Here's how the part is built. I have some questions about the finished solid (model axes, mm). A direction names the side the tool comes from. Round coordinates to 2 decimals unless told otherwise and drop trailing zeros. Write each loop counter-clockwise with the first axis right and the second up, starting at its lowest first coordinate (ties: lowest second). Pieces come first, ordered by that corner, then holes. Notation, with made-up numbers: (70, 38.5) -> (112, 38.5) arc R14 cw to (112, 44.5) -> close; hole circle Ø9 at (15.25, -31.5). An arc over 180 degrees is marked (long way). Answer in a Markdown table with one row per item.
from build123d import *

# Parameters (mm, degrees)
SKETCH_1_W          = 30
SKETCH_1_H          = 50
SKETCH_1_W_2        = 24
SKETCH_1_H_2        = 44
EXTRUDE_1_DEPTH     = 900
SKETCH_2_R          = 10
CUT_EXTRUDE_2_DEPTH = 900
EXTRUDE_2_DEPTH     = 50
SKETCH_4_W          = 30
SKETCH_4_H          = 50
SKETCH_4_W_2        = 24
SKETCH_4_H_2        = 44
EXTRUDE_3_DEPTH     = 15
EXTRUDE_4_DEPTH     = 50


with BuildPart() as part:
    # 草图1 → 凸台-拉伸1 (new body)
    with BuildSketch(Plane.XY):
        with Locations((15, 25)):
            Rectangle(SKETCH_1_W, SKETCH_1_H)
        with Locations((15, 25)):
            Rectangle(SKETCH_1_W_2, SKETCH_1_H_2, mode=Mode.SUBTRACT)
    extrude(amount=EXTRUDE_1_DEPTH)

    # 草图2 → 切除-拉伸2 (cut)
    with BuildSketch(Plane(origin=(0, 50, 0), x_dir=(1, 0, 0), z_dir=(0, 1, 0))):
        with Locations(Location((15, -15, 0), (0, 0, 270))):
            Circle(SKETCH_2_R)
        with BuildLine():
            ThreePointArc((0, -15), (4.393398282, -4.393398282), (15, 0))
            Line((15, 0), (0, 0))
            Line((0, 0), (0, -15))
        make_face()
        with BuildLine():
            Line((30, 0), (15, 0))
            ThreePointArc((15, 0), (25.606601718, -4.393398282), (30, -15))
            Line((30, -15), (30, 0))
        make_face()
    extrude(amount=-CUT_EXTRUDE_2_DEPTH, mode=Mode.SUBTRACT)

    # 草图3 → 凸台-拉伸2 (add)
    with BuildSketch(Plane(origin=(0, 50, 0), x_dir=(1, 0, 0), z_dir=(0, 1, 0))):
        with BuildLine():
            Line((2, -15), (0, -15))
            ThreePointArc((0, -15), (15, 0), (30, -15))
            Line((30, -15), (28, -15))
            ThreePointArc((28, -15), (15, -2), (2, -15))
        make_face()
    extrude(amount=-EXTRUDE_2_DEPTH)

    # 草图4 → 凸台-拉伸3 (add)
    with BuildSketch(Plane.XY.offset(900)):
        with Locations((15, 25)):
            Rectangle(SKETCH_4_W, SKETCH_4_H)
        with Locations((15, 25)):
            Rectangle(SKETCH_4_W_2, SKETCH_4_H_2, mode=Mode.SUBTRACT)
    extrude(amount=EXTRUDE_3_DEPTH)

    # 草图5 → 凸台-拉伸4 (add)
    with BuildSketch(Plane(origin=(0, 50, 0), x_dir=(1, 0, 0), z_dir=(0, 1, 0))):
        with BuildLine():
            Line((-12.2207709, -920.098671199), (-8.128726759, -920.098671199))
            ThreePointArc((-8.128726759, -920.098671199), (15, -914.491908276), (38.128726759, -920.098671199))
            Line((38.128726759, -920.098671199), (42.2207709, -920.098671199))
            ThreePointArc((42.2207709, -920.098671199), (15, -912.491908276), (-12.2207709, -920.098671199))
        make_face()
    extrude(amount=-EXTRUDE_4_DEPTH)


solid = part.part
1) I want a section at A-A, the plane z = 600. List the corners of the cut face in (x, y) for me.
Response:
| item | result |
|---|---|
| outline | (0, 0) -> (30, 0) -> (30, 50) -> (0, 50) -> close; hole (3, 3) -> (27, 3) -> (27, 47) -> (3, 47) -> close |
2) For pin 1 (5 mm diameter, centred on x = 21.5, y = 18.5, fed in from +Z); pin 2 (23 mm diameter, centred on x = 15, z = 15, fed in from -Y); pin 3 (2 mm diameter, centred on x = 11, y = 18, fed in from +Z); pin 4 (12 mm diameter, centred on y = 16.5, z = 594.5, fed in from +X), each with a flat end and sliding along its axis, tell me the tip position at first contact or that it passes through.
Response:
| item | result |
|---|---|
| pin 1 | stops at z = 915.3 |
| pin 2 | stops at y = 0 |
| pin 3 | stops at z = 914.74 |
| pin 4 | stops at x = 30 |
3) We'd pull the mould along Y, two halves only. Please class faces 1 (the face through (15, 0, 454)), 2 (the face through (15, 3, 452)): +Y half, -Y half, draft (parallel to the pull), parting line (faces both ways), or undercut.
Response:
| item | result |
|---|---|
| face 1 | -Y half |
| face 2 | undercut |
4) Which directions (+Z, -Z, +X, -X, +Y, -Y) give clear straight access to the entire face, cutting with the end or side of a thin tool? Please do faces 3 (the face through (0, 25, 459)), 4 (the face through (18, 48.52, 24.54)), 5 (the face through (15.169, 25.308, 912.492)), 6 (the face through (30, 25, 459)).
Response:
| item | result |
|---|---|
| face 3 | -Z, -X, +Y, -Y |
| face 4 | +Y, -Y |
| face 5 | none |
| face 6 | -Z, +X, +Y, -Y |
5) I want a section at B-B, the plane y = 15.5. List the corners of the cut face in (x, z) for me, and give its area (3 significant figures).
Response:
| item | result |
|---|---|
| outline | (-12.22, 920.1) arc R52.51 ccw to (0, 914.68) -> (0, 15) arc R15 ccw to (30, 15) -> (30, 914.68) arc R52.51 ccw to (42.22, 920.1) -> (38.13, 920.1) arc R50.51 cw to (-8.13, 920.1) -> close; hole (3, 10) arc R13 ccw to (27, 10) -> (27, 913.88) arc R52.51 cw to (3, 913.88) -> close |
| area | 5,600 mm^2 |
6) I need wall thicknesses on line 1 (X direction, y = 32.5, z = 603); line 2 (Y direction, x = 10, z = 633.5); line 3 (X direction, y = 0.8, z = 15). Which ranges of each line are inside material? Lowest first, please. Write a range as [from, to].
Response:
| item | result |
|---|---|
| line 1 | x = [0, 3], [27, 30] |
| line 2 | y = [0, 3], [47, 50] |
| line 3 | x = [0, 5], [25, 30] |
